from build123d import *

# Parameters (mm, degrees)
PIN_PROFILE_SKETCH_W   = 25
PIN_PROFILE_SKETCH_H   = 7.5
PIN_PROFILE_SKETCH_W_2 = 125
PIN_PROFILE_SKETCH_H_2 = 20


with BuildPart() as part:
    # Pin Profile Sketch → Pin Body Revolve (revolve)
    with BuildSketch(Plane.XY):
        with Locations((-15.5, 3.75)):
            Rectangle(PIN_PROFILE_SKETCH_W, PIN_PROFILE_SKETCH_H)
        with Locations((62.5, 10)):
            Rectangle(PIN_PROFILE_SKETCH_W_2, PIN_PROFILE_SKETCH_H_2)
        Polygon((-3, 0), (0, 0), (0, 20), (-3, 17), (-3, 7.5), align=None)
        Polygon((125, 0), (135, 0), (135, 30), (125, 20), align=None)
        Polygon((135, 0), (145, 0), (145, 30), (135, 40), (135, 30), align=None)
    revolve(axis=Axis((213.258902513, 0, 0), (-1, 0, 0)))


solid = part.part
The model under review builds one solid part; all positions refer to its coordinate system, in mm. A direction names the side the tool comes from. Coordinates: 2 decimals unless noted, no trailing zeros. Write each loop counter-clockwise with the first axis right and the second up, starting at its lowest first coordinate (ties: lowest second). Pieces come first, ordered by that corner, then holes. Notation, with made-up numbers: (88.5, 30.5) - (110.5, 30.5) arc R17 ccw to (110.5, 63.5) - close; hole circle Ø7 at (-4, 11). An arc over 180 degrees is marked (long way). Answer as CSV lines item,"result".
(1) We need section A-A (y = 0). Give the boundary of the cut face in (x, z).
Data:
outline,"(-28, -7.5) - (-3, -7.5) - (-3, -17) - (0, -20) - (125, -20) - (135, -30) - (135, -40) - (145, -30) - (145, 30) - (135, 40) - (135, 30) - (125, 20) - (0, 20) - (-3, 17) - (-3, 7.5) - (-28, 7.5) - close"
(2) For line 1 along Z through (x, y) = (31, 1); line 2 along X through (y, z) = (27, 10.5), list the stretches that pass through material, from the lowest coordinate up. Write a range as [from, to].
Data:
line 1,"z = [-19.97, 19.97]"
line 2,"x = [133.97, 145]"
(3) Clearance check with flat-ended pins moving along their axes: pin 1 Ø24 at (y, z) = (17, -3.5) entering from -X; pin 2 Ø6 at (y, z) = (15.5, -20.5) entering from -X; pin 3 Ø6 at (x, z) = (-4, 16.5) entering from +Y; pin 4 Ø8 at (y, z) = (21.5, 10.5) entering from -X. State where each tip first meets the part, or that it passes through.
Data:
pin 1,"stops at x = -28"
pin 2,"stops at x = 127.7"
pin 3,"stops at y = 11.07"
pin 4,"stops at x = -0.07"
(4) We need section C-C (x = 37.5). Give the boundary of the cut face in (y, z).
Data:
outline,"circle Ø40 at (0, 0)"
(5) Tool access review of faces 1 (the conical face through (144.374, -3.987, -30.365)), 2 (the flat face through (-3, 7, 4)): name each direction out of +Z, -Z, +X, -X, +Y, -Y from which nothing blocks a thin tool from reaching the whole face with its end or side.
Data:
face 1,"+X"
face 2,"-X"
